from build123d import *

# Parameters (mm, degrees)
SKETCH_1_W      = 20
SKETCH_1_H      = 20
SKETCH_1_W_2    = 10
SKETCH_1_H_2    = 10
EXTRUDE_1_DEPTH = 10
SKETCH_2_R      = 5
EXTRUDE_2_DEPTH = 10


with BuildPart() as part:
    # 草图1 → 凸台-拉伸1 (new, symmetric)
    with BuildSketch(Plane.XY):
        with Locations((5, 5)):
            Rectangle(SKETCH_1_W, SKETCH_1_H)
        with Locations((5, 5)):
            Rectangle(SKETCH_1_W_2, SKETCH_1_H_2, mode=Mode.SUBTRACT)
    extrude(amount=EXTRUDE_1_DEPTH, both=True)

    # 草图2 → 凸台-拉伸2 (add)
    with BuildSketch(Plane.XZ.offset(5)):
        with Locations(Location((5, 0, 0), (0, 0, 90))):
            Circle(SKETCH_2_R)
    extrude(amount=EXTRUDE_2_DEPTH)


solid = part.part
Part model, mm, in its own coordinate system. A direction names the side the tool comes from. Coordinates: 2 decimals unless noted, no trailing zeros. Order: outer loops, then holes, each group sorted by start corner. A loop starts at its lowest first (then second) coordinate and runs counter-clockwise, first axis right, second up.
(1) Slice it at B-B, the plane z = -7.25. Write the cut outline in (x, y), and give its area (3 significant figures).
Check sheet entries:
outline: (-5, -5) - (15, -5) - (15, 15) - (-5, 15) - close; hole (0, 0) - (10, 0) - (10, 10) - (0, 10) - close
area: 300 mm2
(2) Probe L1, parallel to X at y = 9.5, z = -0.5; L2, parallel to Y at x = 9, z = 0. List the from-to ranges inside material, lowest first.
Check sheet entries:
L1: x = -5 to 0, 10 to 15
L2: y = -15 to 0, 10 to 15
(3) Slice it at C-C, the plane x = 5. Write the cut outline in (y, z), and give its area (3 significant figures).
Check sheet entries:
outline: (-15, -5) - (-5, -5) - (-5, -10) - (0, -10) - (0, 10) - (-5, 10) - (-5, 5) - (-15, 5) - close; (10, -10) - (15, -10) - (15, 10) - (10, 10) - close
area: 300 mm2
(4) Slice it at A-A, the plane y = 3. Write the cut outline in (x, z).
Check sheet entries:
outline: (-5, -10) - (0, -10) - (0, 10) - (-5, 10) - close; (10, -10) - (15, -10) - (15, 10) - (10, 10) - close
(5) Pin check, flat tips, straight feed: pin 1 Ø8 at (x, y) = (-1, -9.5) entering from -Z; pin 2 Ø5 at (x, z) = (-3, 5.5) entering from -Y; pin 3 Ø6 at (x, y) = (4.5, -7.5) entering from +Z. Stop position of each tip, or through.
Check sheet entries:
pin 1: stops at z = -4.58
pin 2: stops at y = -5
pin 3: stops at z = 10
(6) Tool access for faces 1 (the face through (5, -15, 0)), 2 (the face through (5, 10, 0)), 3 (the face through (9.436, -9.93, 2.307)): list every direction of +Z, -Z, +X, -X, +Y, -Y with a clear straight run to the whole face (end or side of a thin tool).
Check sheet entries:
face 1: +Z, -Z, +X, -X, -Y
face 2: +Z, -Z
face 3: -Y
(7) Pull direction Y, two halves, no side cores. Call faces 4 (the face through (5, 15, 0)), 5 (the face through (3, -5, 5)), 6 (the face through (5, 12, -10)), 7 (the face through (0, 5, 0)): pulls with the +Y half, pulls with the -Y half, needs draft (parallel to the pull), parting line crosses it, or undercut.
Check sheet entries:
face 4: pulls with the +Y half
face 5: pulls with the -Y half
face 6: needs draft
face 7: undercut
(8) Slice it at D-D, the plane z = 0. Write the cut outline in (x, y), and give its area (3 significant figures).
Check sheet entries:
outline: (-5, -5) - (0, -5) - (0, -15) - (10, -15) - (10, -5) - (15, -5) - (15, 15) - (-5, 15) - close; hole (0, 0) - (10, 0) - (10, 10) - (0, 10) - close
area: 400 mm2
